Answer from the drawing. Dimensions are ordinates in mm from the lowest x, y and z of the part. Coordinates: 2 decimals unless noted, no trailing zeros. Order: outer loops, then holes, each group sorted by start corner. A loop starts at its lowest first (then second) coordinate and runs counter-clockwise, first axis right, second up. Notation, with made-up numbers: (-20, 50.25) -> (19, 50.25) arc R28 ccw to (19, 80.25) -> close; hole circle Ø5 at (58, -28.75). An arc over 180 degrees is marked (long way). Answer as a JSON object with one key per item and string values. Group by question number.
1) Section B-B on z = 2 is taken. Determine the outline of the cut face in (x, y).
2) Consider L1, parallel to Y at x = 32.5, z = 5.5; L2, parallel to X at y = 56, z = 2; L3, parallel to X at y = 57.5, z = 5.25 (1 decimal). Determine where each line is inside the solid, lowest interval first.
3) Section C-C on y = 53 is taken. Determine the outline of the cut face in (x, z).
4) Determine the mould class of the marked faces 1, 2, 3 and 4 for opening direction X: released by +X, released by -X, zero draft, split by the parting line, or undercut.
5) Section A-A on x = 32.5 is taken. Determine the outline of the cut face in (y, z), and give its area (3 significant figures).
6) Section D-D on y = 7.5 is taken. Determine the outline of the cut face in (x, z), and give its area (3 significant figures).
7) Given pin 1 (1.5 mm diameter, centred on y = 46, z = 6, fed in from -X); pin 2 (2 mm diameter, centred on y = 18, z = 6, fed in from -X); pin 3 (6 mm diameter, centred on x = 49.5, y = 51.5, fed in from -Z); pin 4 (3 mm diameter, centred on y = 17.5, z = 2, fed in from -X), each flat-ended and moving along its own axis, determine where each tip first touches the part or whether it passes through.
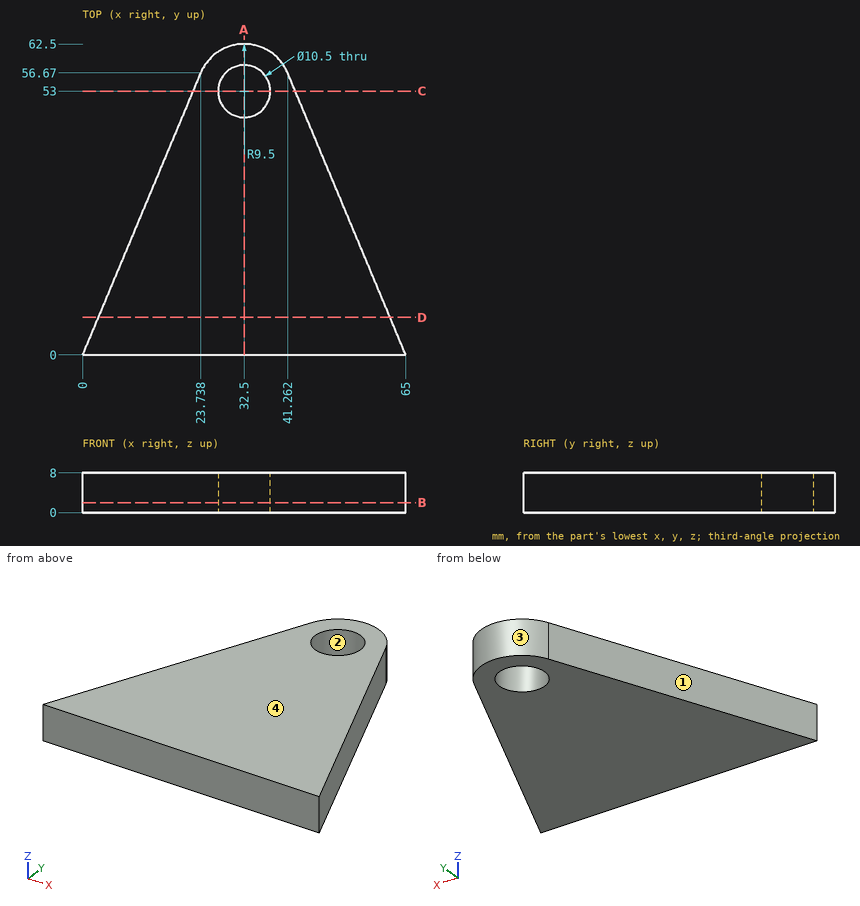
Worked answers:
{
 "1": {"outline": "(0, 0) -> (65, 0) -> (41.26, 56.67) arc R9.5 ccw to (23.74, 56.67) -> close; hole circle Ø10.5 at (32.5, 53)"},
 "2": {"L1": "y = 0 to 47.75, 58.25 to 62.5", "L2": "x = 23.46 to 28.19, 36.81 to 41.54", "L3": "x = 24.1 to 29.8, 35.2 to 40.9"},
 "3": {"outline": "(22.2, 0) -> (27.25, 0) -> (27.25, 8) -> (22.2, 8) -> close; (37.75, 0) -> (42.8, 0) -> (42.8, 8) -> (37.75, 8) -> close"},
 "4": {"face 1": "released by -X", "face 2": "undercut", "face 3": "split by the parting line", "face 4": "zero draft"},
 "5": {"outline": "(0, 0) -> (47.75, 0) -> (47.75, 8) -> (0, 8) -> close; (58.25, 0) -> (62.5, 0) -> (62.5, 8) -> (58.25, 8) -> close", "area": "416 mm²"},
 "6": {"outline": "(3.14, 0) -> (61.86, 0) -> (61.86, 8) -> (3.14, 8) -> close", "area": "470 mm²"},
 "7": {"pin 1": "stops at x = 18.95", "pin 2": "stops at x = 7.12", "pin 3": "passes through", "pin 4": "stops at x = 6.7"}
}
